from build123d import *

# Parameters (mm, degrees)
PIVOT_TUBE_SKETCH_R         = 15
PIVOT_TUBE_SKETCH_R_2       = 7.5
PIVOT_TUBE_30X_15_DEPTH     = 40
ARM_WEB_20MM_DEPTH          = 10
RING_HUB_SKETCH_R           = 60
RING_HUB_SKETCH_R_2         = 50
RING_HUB_120X_100_DEPTH     = 15
ARM_LIGHTENING_POCKET_DEPTH = 230.401394939


with BuildPart() as part:
    # Pivot Tube Sketch → Pivot Tube Ø30xØ15 (new, symmetric)
    with BuildSketch(Plane(origin=(0, 0, 0), x_dir=(0, 0, -1), z_dir=(1, 0, 0))):
        Circle(PIVOT_TUBE_SKETCH_R)
        Circle(PIVOT_TUBE_SKETCH_R_2, mode=Mode.SUBTRACT)
    extrude(amount=PIVOT_TUBE_30X_15_DEPTH, both=True)

    # Arm Web Sketch → Arm Web 20mm (add, symmetric)
    with BuildSketch(Plane(origin=(0, 0, 0), x_dir=(1, 0, 0), z_dir=(0, 1, 0))):
        with BuildLine():
            Line((-57.295515099, 142.189218166), (-16.443257741, 10.771566203))
            Line((-16.443257741, 10.771566203), (19.870461321, 10.771566203))
            Line((19.870461321, 10.771566203), (57.703615224, 143.559416372))
            ThreePointArc((57.703615224, 143.559416372), (0.714840688, 100.004258461), (-57.295515099, 142.189218166))
        make_face()
    extrude(amount=ARM_WEB_20MM_DEPTH, both=True)

    # Ring Hub Sketch → Ring Hub Ø120xØ100 (add, symmetric)
    with BuildSketch(Plane(origin=(0, 0, 0), x_dir=(1, 0, 0), z_dir=(0, 1, 0))):
        with Locations(Location((0, 160, 0), (0, 0, 270))):
            Circle(RING_HUB_SKETCH_R)
        with Locations(Location((0, 160, 0), (0, 0, 270))):
            Circle(RING_HUB_SKETCH_R_2, mode=Mode.SUBTRACT)
    extrude(amount=RING_HUB_120X_100_DEPTH, both=True)

    # Arm Pocket Sketch → Arm Lightening Pocket (cut, through all)
    with BuildSketch(Plane(origin=(0, 10, 0), x_dir=(1, 0, 0), z_dir=(0, 1, 0))):
        with BuildLine():
            Line((-13.0584069, 38.71360492), (16.320169694, 38.71360492))
            ThreePointArc((16.320169694, 38.71360492), (19.277035427, 39.681614712), (21.088991166, 42.210826904))
            Line((21.088991166, 42.210826904), (34.445867452, 84.596700091))
            ThreePointArc((34.445867452, 84.596700091), (33.039335954, 89.800154549), (27.725249342, 90.702791032))
            ThreePointArc((27.725249342, 90.702791032), (0.71662682, 85.149887641), (-26.34110962, 90.458307872))
            ThreePointArc((-26.34110962, 90.458307872), (-31.704790858, 89.453148124), (-32.954629394, 84.141149802))
            Line((-32.954629394, 84.141149802), (-17.761840528, 42.017222858))
            ThreePointArc((-17.761840528, 42.017222858), (-15.932262297, 39.622033687), (-13.0584069, 38.71360492))
        make_face()
    extrude(amount=-ARM_LIGHTENING_POCKET_DEPTH, mode=Mode.SUBTRACT)


solid = part.part
Could you check a few things on this model? Use its own coordinates, in mm. A direction names the side the tool comes from. Give positions to 0.01 mm unless a question says otherwise; leave off trailing zeros. Order: outer loops, then holes, each group sorted by start corner. A loop starts at its lowest first (then second) coordinate and runs counter-clockwise, first axis right, second up. Notation, with made-up numbers: (75.5, 57.25) - (91.5, 57.25) arc R30 cw to (91.5, 86.25) - close; hole circle Ø9 at (60.25, 75). An arc over 180 degrees is marked (long way). One line per question, with ' | ' between items. Start each with the question number.
Item 1: I'm going to push flat-ended pins straight in: pin 1 Ø8 at (x, y) = (-19, -0.5) entering from -Z; pin 2 Ø4 at (x, z) = (-1.5, -95) entering from +Y; pin 3 Ø10 at (y, z) = (-6.5, -50.5) entering from -X. Where does each tip first touch, or does it pass through?
Item 2: I want a section at B-B on x = 0. Write out the boundary of the cut face in (y, z).
Item 3: I want a section at D-D on z = -160. Write out the boundary of the cut face in (x, y).
Item 4: Thinking about a two-plate mould opening in X: for faces 6 (the cylindrical face through (33.098, 0.14, -89.746)), 7 (the cylindrical face through (0.56, 0.66, 14.985)), 8 (the flat face through (38.58, 0.14, -76.44)), which applies, pulls with the +X half, pulls with the -X half, needs draft (parallel to the pull), parting line crosses it, or undercut?
Item 5: For faces 1 (the cylindrical face through (-15.97, 0.14, -39.65)), 2 (the flat face through (-40, 7, 4)), 3 (the cylindrical face through (-0.56, 0.33, 7.493)), 4 (the flat face through (40, 7, 4)), 5 (the flat face through (45, 15, -183)), which set-ups out of +Z, -Z, +X, -X, +Y, -Y let a thin tool reach every point of the face, with its end or its side?
Item 6: I want a section at C-C on y = -2.5. Write out the boundary of the cut face in (x, z), then the cut area to 3 significant figures.
Item 7: I need wall thicknesses on probe 1 along X at (y, z) = (-2, -160); probe 2 along Z at (x, y) = (1, 6.5); probe 3 along Z at (x, y) = (19.5, -6.5). Which ranges of each line are inside material? Lowest first, please. Write a range as [from, to].
Item 8: I want a section at A-A on z = 0. Write out the boundary of the cut face in (x, y).
Verdict:
1) pin 1: z = -218.09 | pin 2: y = 10 | pin 3: x = -30.35
2) outline: (-15, -220) - (15, -220) - (15, -210) - (-15, -210) - close; (-15, -110) - (15, -110) - (15, -100) - (10, -100) - (10, -85.15) - (-10, -85.15) - (-10, -100) - (-15, -100) - close; (-10, -38.71) - (10, -38.71) - (10, -11.18) arc R15 ccw (long way) to (-10, -11.18) - close; hole circle Ø15 at (0, 0)
3) outline: (-60, -15) - (-50, -15) - (-50, 15) - (-60, 15) - close; (50, -15) - (60, -15) - (60, 15) - (50, 15) - close
4) face 6: undercut | face 7: needs draft | face 8: pulls with the +X half
5) face 1: +Y, -Y | face 2: +Z, -X, +Y, -Y | face 3: +X, -X | face 4: +Z, +X, +Y, -Y | face 5: +Z, -Z, +X, -X, +Y
6) outline: (-57.3, -142.19) arc R60 ccw (long way) to (57.7, -143.56) - (21.02, -14.79) - (40, -14.79) - (40, -7.07) - (-40, -7.07) - (-40, -14.79) - (-17.69, -14.79) - close; (-40, 7.07) - (40, 7.07) - (40, 14.79) - (-40, 14.79) - close; hole circle Ø100 at (0, -160); hole (-32.95, -84.14) arc R5 ccw to (-26.34, -90.46) arc R70 cw to (27.73, -90.7) arc R5 ccw to (34.45, -84.6) - (21.09, -42.21) arc R5 ccw to (16.32, -38.71) - (-13.06, -38.71) arc R5 ccw to (-17.76, -42.02) - close | area: 8,320 mm^2
7) probe 1: [-60, -50], [50, 60] | probe 2: [-219.99, -209.99], [-110.01, -85.15], [-38.71, -3.74], [3.74, 13.52] | probe 3: [-216.74, -206.04], [-113.96, -87.81], [-39.86, -3.74], [3.74, 13.52]
8) outline: (-40, -15) - (40, -15) - (40, -7.5) - (-40, -7.5) - close; (-40, 7.5) - (40, 7.5) - (40, 15) - (-40, 15) - close
